Print and shaded views of the part. All mm, measured from the part's lowest x, y and z. Coordinates: 2 decimals unless noted, no trailing zeros. Order: outer loops, then holes, each group sorted by start corner. A loop starts at its lowest first (then second) coordinate and runs counter-clockwise, first axis right, second up. Notation, with made-up numbers: (-34, 11) -> (-30, 11) arc R30 cw to (-30, 43) -> close; hole circle Ø5 at (24.5, -26). An arc over 180 degrees is marked (long way). Write item = value, one per line. Start each with the question number.
Q1. Wall check: line 1 (X direction, y = 1.9, z = 1.5); line 2 (Y direction, x = 21.5, z = 1.1). Give the ranges that are in metal, low to high. Write a range as from..to.
Q2. Cut at A-A, the plane x = 6. List the corners of the cut face in (y, z), plus the area to 3 significant figures.
Q3. Flat gauge pin, fed straight in: pin 1 (6 mm diameter, centred on x = 23.5, y = 20, fed in from -Z). Where does the tip first touch, or does it go through?
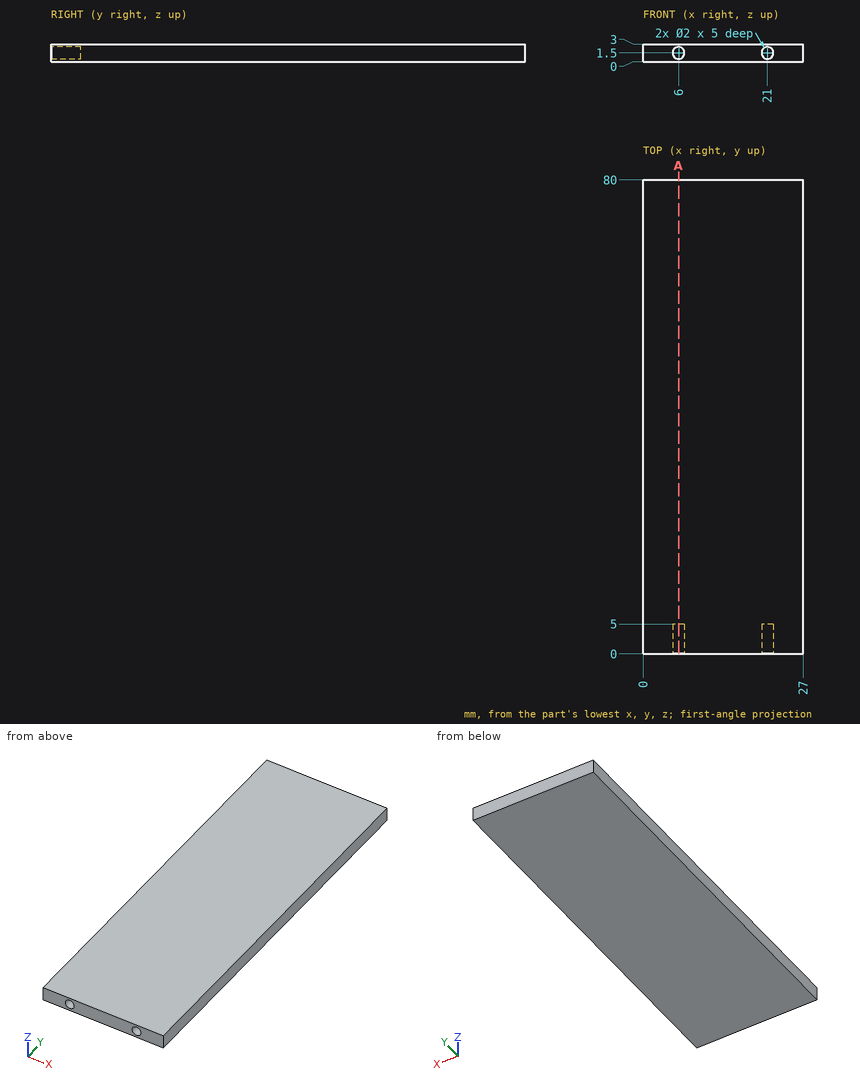
Here are the results:
q1.line_1 = 0..5, 7..20, 22..27
q1.line_2 = 5..80
q2.outline = (0, 0) -> (80, 0) -> (80, 3) -> (0, 3) -> (0, 2.5) -> (5, 2.5) -> (5, 0.5) -> (0, 0.5) -> close
q2.area = 230 mm²
q3.pin_1 = 0
